The listing builds one solid part. Answer for the finished solid, in the listing's coordinates (mm). Face numbers are marked on the shaded views. A direction names the side the tool comes from. Round coordinates to 2 decimals unless told otherwise and drop trailing zeros. Order: outer loops, then holes, each group sorted by start corner. A loop starts at its lowest first (then second) coordinate and runs counter-clockwise, first axis right, second up. Notation, with made-up numbers: M 50,73.5 L 91,73.5 A29 cw 91,96.5 Z; hole C 35.5,26.25 d4. An arc over 180 degrees is marked long. Put each result on its own line as item: value. Start each with the question number.
1. The part is cut by section A-A (x = -1). Give the vertices of the cut face in (y, z), then the cut area to 3 significant figures.
2. The part is cut by section C-C (z = 79). Give the vertices of the cut face in (x, y).
3. Consider line 1 (Y direction, x = -16, z = 226); line 2 (Y direction, x = 16.5, z = 259.5). Determine where each line is inside the solid, lowest interval first.
4. Which of the six approach directions +Z, -Z, +X, -X, +Y, -Y give full straight-line access (tool end or side, diameter ignored) to the marked faces 1 and 2?
5. This flat-tipped pin is pushed along its axis until it touches: pin 1 Ø10 at (x, y) = (-8.5, 7.5) entering from -Z. Where does it stop, or does it pass through?
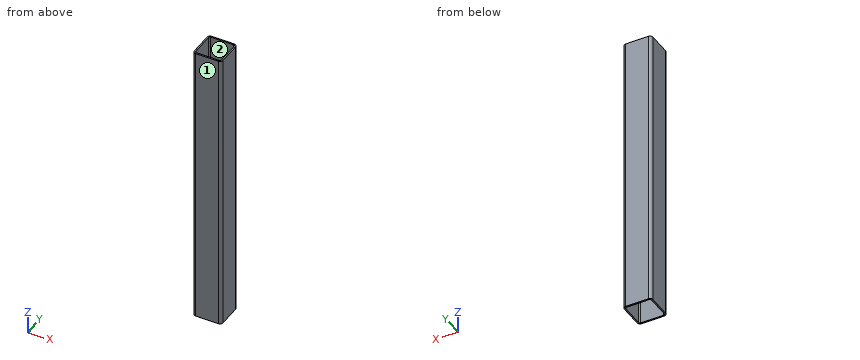
from build123d import *

# Parameters (mm, degrees)
SKETCH1_W           = 40
SKETCH1_H           = 40
SKETCH1_W_2         = 36
SKETCH1_H_2         = 36
BOSS_EXTRUDE1_DEPTH = 403
FILLET1_R           = 2
FILLET2_R           = 4


with BuildPart() as part:
    # Sketch1 → Boss-Extrude1 (new body)
    with BuildSketch(Plane.XY):
        Rectangle(SKETCH1_W, SKETCH1_H)
        Rectangle(SKETCH1_W_2, SKETCH1_H_2, mode=Mode.SUBTRACT)
    extrude(amount=BOSS_EXTRUDE1_DEPTH)

    # Fillet1
    fillet1_edges = [part.edges().sort_by_distance(p)[0] for p in [
        (18, -18, 201.5),
        (18, 18, 201.5),
        (-18, 18, 201.5),
        (-18, -18, 201.5),
    ]]
    fillet(fillet1_edges, radius=FILLET1_R)

    # Fillet2
    fillet2_edges = [part.edges().sort_by_distance(p)[0] for p in [
        (20, -20, 201.5),
        (-20, -20, 201.5),
        (-20, 20, 201.5),
        (20, 20, 201.5),
    ]]
    fillet(fillet2_edges, radius=FILLET2_R)


solid = part.part
Resolved:
1. outline: M -20,0 L -18,0 L -18,403 L -20,403 Z; M 18,0 L 20,0 L 20,403 L 18,403 Z
1. area: 1,610 mm2
2. outline: M -20,-16 A4 ccw -16,-20 L 16,-20 A4 ccw 20,-16 L 20,16 A4 ccw 16,20 L -16,20 A4 ccw -20,16 Z; hole M -18,-16 A2 ccw -16,-18 L 16,-18 A2 ccw 18,-16 L 18,16 A2 ccw 16,18 L -16,18 A2 ccw -18,16 Z
3. line 1: -20 to -18, 18 to 20
3. line 2: -19.97 to -17.94, 17.94 to 19.97
4. face 1: +Z, -Z, +X, -X, -Y
4. face 2: +Z, -Z
5. pin 1: through
